Verification items for the finished model (mm, model axes). Face numbers are marked on the shaded views. A direction names the side the tool comes from. Round coordinates to 2 decimals unless told otherwise and drop trailing zeros. Order: outer loops, then holes, each group sorted by start corner. A loop starts at its lowest first (then second) coordinate and runs counter-clockwise, first axis right, second up. Notation, with made-up numbers: M 4.25,2.5 L 36.25,2.5 A13 cw 36.25,18.5 Z; hole C 30.5,20.25 d8. An arc over 180 degrees is marked long. Write item = value, one per line. Start each with the question number.
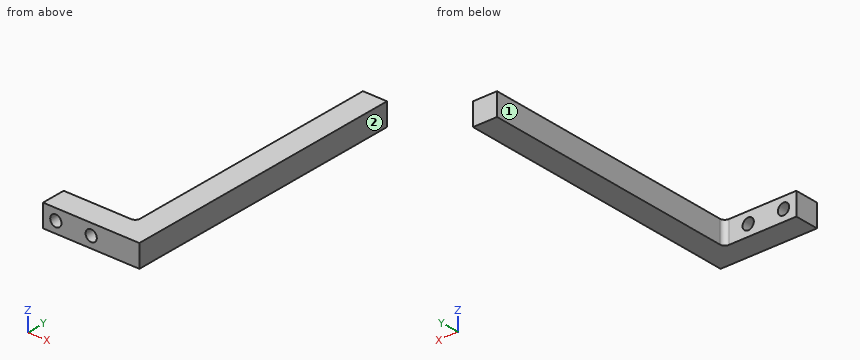
from build123d import *

# Parameters (mm, degrees)
EXTRUDE_1_DEPTH     = 7
FILLET_1_R          = 3
CUT_EXTRUDE_1_REACH = 177.71
SKETCH_3_R          = 3.5


with BuildPart() as part:
    # 草图1 → 凸台-拉伸1 (new, symmetric)
    with BuildSketch(Plane.XY):
        Polygon((0, 180), (-15, 180), (-15, 15), (-60, 15), (-60, 0), (0, 0), align=None)
    extrude(amount=EXTRUDE_1_DEPTH, both=True)

    # 圆角1
    fillet_1_edges = [part.edges().sort_by_distance(p)[0] for p in [
        (-15, 15, 0),
    ]]
    fillet(fillet_1_edges, radius=FILLET_1_R)

    # 草图3 → 切除-拉伸1 (cut, up to next)
    with BuildSketch(Plane(origin=(0, 15, 0), x_dir=(1, 0, 0), z_dir=(0, 1, 0)), mode=Mode.PRIVATE) as cut_extrude_1_sk1:
        with Locations(Location((-52, 0, 0), (0, 0, 180))):
            Circle(SKETCH_3_R)
    cut_extrude_1_tool1 = extrude(cut_extrude_1_sk1.sketch, amount=-CUT_EXTRUDE_1_REACH, mode=Mode.PRIVATE) & part.part
    # 草图3 → 切除-拉伸1 (cut, up to next)
    with BuildSketch(Plane(origin=(0, 15, 0), x_dir=(1, 0, 0), z_dir=(0, 1, 0)), mode=Mode.PRIVATE) as cut_extrude_1_sk2:
        with Locations(Location((-30, 0, 0), (0, 0, 180))):
            Circle(SKETCH_3_R)
    cut_extrude_1_tool2 = extrude(cut_extrude_1_sk2.sketch, amount=-CUT_EXTRUDE_1_REACH, mode=Mode.PRIVATE) & part.part
    add(cut_extrude_1_tool1.solids().sort_by_distance((-52, 15, 0))[0], mode=Mode.SUBTRACT)
    add(cut_extrude_1_tool2.solids().sort_by_distance((-30, 15, 0))[0], mode=Mode.SUBTRACT)


solid = part.part
1) Scan lines: probe 1 along Z at (x, y) = (-52, 6.75); probe 2 along Y at (x, z) = (-20, -3); probe 3 along X at (y, z) = (104, 0.5). Record each from-to range of solid material in increasing order.
2) Cross-section at A-A, the plane x = -30. Enter the section's corners in (y, z).
3) Cross-section at B-B, the plane z = 0. Enter the section's corners in (x, y), then the cut area to 3 significant figures.
4) Gauge pin test, flat ends, axial feed: P1, Ø4, axis at x = -28.5, z = -1, coming from the +Y side; P2, Ø4, axis at x = -52, z = 0, coming from the +Y side; P3, Ø4, axis at y = 72.5, z = -3, coming from the -X side. Record the tip position at first contact, or that the pin passes through.
5) Cross-section at C-C, the plane y = 43.5. Enter the section's corners in (x, z).
6) Cross-section at D-D, the plane x = -51. Enter the section's corners in (y, z).
7) Access from +Z, -Z, +X, -X, +Y, -Y to the whole of each face (thin tool, end or side, straight path). Record for the marked faces 1 and 2.
Geometry results:
q1.probe_1 = -7 to -3.5, 3.5 to 7
q1.probe_2 = 0 to 15
q1.probe_3 = -15 to 0
q2.outline = M 0,-7 L 15,-7 L 15,-3.5 L 0,-3.5 Z; M 0,3.5 L 15,3.5 L 15,7 L 0,7 Z
q3.outline = M -60,0 L -55.5,0 L -55.5,15 L -60,15 Z; M -48.5,0 L -33.5,0 L -33.5,15 L -48.5,15 Z; M -26.5,0 L 0,0 L 0,180 L -15,180 L -15,18 A3 cw -18,15 L -26.5,15 Z
q3.area = 3,170 mm^2
q4.P1 = 15
q4.P2 = through
q4.P3 = -15
q5.outline = M -15,-7 L 0,-7 L 0,7 L -15,7 Z
q6.outline = M 0,-7 L 15,-7 L 15,-3.35 L 0,-3.35 Z; M 0,3.35 L 15,3.35 L 15,7 L 0,7 Z
q7.face_1 = +Z, -Z, -X, +Y
q7.face_2 = +Z, -Z, +X, +Y, -Y
